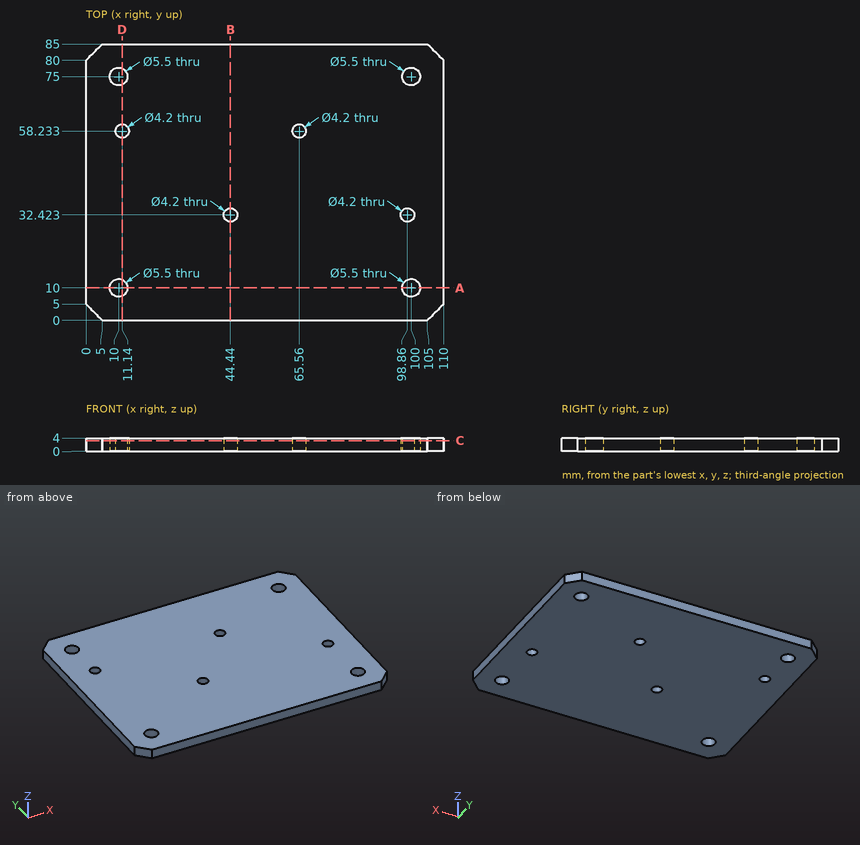
The figure shows three views and two pictorial views of one solid part (mm, origin at its lowest corner). Answer the questions. Coordinates: 2 decimals unless noted, no trailing zeros. Loops run counter-clockwise (first coordinate to the right, second up) from the corner with the lowest first, then second, coordinate; pieces in that order, holes last. Notation, with made-up numbers: (87.25, -3.75) - (125.25, -3.75) arc R28 ccw to (125.25, 19.25) - close; hole circle Ø3 at (85.5, -20.75). An arc over 180 degrees is marked (long way). Use a Markdown table: item, result. Add a question column.
1) Given pin 1 (4 mm diameter, centred on x = 98.86, y = 32.42, fed in from +Z), flat-ended and moving along its own axis, determine where the tip first touches the part or whether it passes through.
2) The part is cut by section C-C, the plane z = 3.3. State how many separate pieces and enclosed holes the cut face has, and give its area (3 significant figures).
3) Find the intervals of material crossed by line 1 (Y direction, x = 98.86, z = 2.6); line 2 (Y direction, x = 44.44, z = 1.2); line 3 (Y direction, x = 11.5, z = 1.35) (1 decimal), in increasing order.
4) The part is cut by section A-A, the plane y = 10. Give the vertices of the cut face in (x, z).
5) The part is cut by section D-D, the plane x = 11.14. Give the vertices of the cut face in (y, z), and give its area (3 significant figures).
6) The part is cut by section B-B, the plane x = 44.44. Give the vertices of the cut face in (y, z), and give its area (3 significant figures).
Here are the results:
| question | item | result |
|---|---|---|
| 1 | pin 1 | passes through |
| 2 | separate pieces | 1 |
| 2 | enclosed holes | 8 |
| 2 | area | 9,150 mm^2 |
| 3 | line 1 | y = 0 to 7.5, 12.5 to 30.32, 34.52 to 72.5, 77.5 to 85 |
| 3 | line 2 | y = 0 to 30.32, 34.52 to 85 |
| 3 | line 3 | y = 0 to 7.7, 12.3 to 56.2, 60.3 to 72.7, 77.3 to 85 |
| 4 | outline | (0, 0) - (7.25, 0) - (7.25, 4) - (0, 4) - close; (12.75, 0) - (97.25, 0) - (97.25, 4) - (12.75, 4) - close; (102.75, 0) - (110, 0) - (110, 4) - (102.75, 4) - close |
| 5 | outline | (0, 0) - (7.5, 0) - (7.5, 4) - (0, 4) - close; (12.5, 0) - (56.13, 0) - (56.13, 4) - (12.5, 4) - close; (60.33, 0) - (72.5, 0) - (72.5, 4) - (60.33, 4) - close; (77.5, 0) - (85, 0) - (85, 4) - (77.5, 4) - close |
| 5 | area | 283 mm^2 |
| 6 | outline | (0, 0) - (30.32, 0) - (30.32, 4) - (0, 4) - close; (34.52, 0) - (85, 0) - (85, 4) - (34.52, 4) - close |
| 6 | area | 323 mm^2 |
